Can you work these out from the model? Positions are in its coordinate system, mm. Face numbers are marked on the shaded views. A direction names the side the tool comes from. Give positions to 0.01 mm unless a question says otherwise; leave off trailing zeros. Write each loop counter-clockwise with the first axis right and the second up, starting at its lowest first coordinate (ties: lowest second). Pieces come first, ordered by that corner, then holes. Notation, with made-up numbers: (31, 23) -> (42, 23) arc R24 cw to (42, 35) -> close; hole circle Ø1 at (47.5, 84.5). An arc over 180 degrees is marked (long way). Answer as CSV lines item,"result". Start each with the question number.
1. If we section it at A-A on x = 18.5: Write out the boundary of the cut face in (y, z).
2. On a 3-axis mill with a long thin cutter (end or side, diameter ignored), from which of +Z, -Z, +X, -X, +Y, -Y can I reach the whole of each face in a straight line? I mean the marked faces 1, 2 and 3. Say none if no direction works.
3. I need wall thicknesses on line 1 (Y direction, x = 53.5, z = 4.25); line 2 (X direction, y = 33.5, z = 3.1); line 3 (Y direction, x = 41.5, z = 1.7). Which ranges of each line are inside material? Lowest first, please. Write a range as [from, to].
4. If we mould it in two halves opening along X, with no side actions, what happens to the marked faces 4, 5 and 6? For each: pulls with the +X half, pulls with the -X half, needs draft (parallel to the pull), parting line crosses it, or undercut.
5. If we section it at B-B on z = 7: Count the separate pieces of the cut face and the enclosed holes in it, plus the area to 3 significant figures.
6. I'm going to push flat-ended pins straight in: P1, Ø3, axis at x = 54.5, y = 32.5, coming from the -Z side; P2, Ø2.5, axis at x = 41.5, y = 37, coming from the +Z side; P3, Ø2.5, axis at x = 18, y = 38, coming from the +Z side. Where does each tip first touch, or does it pass through?
7. If we section it at C-C on y = 12.5: Write out the boundary of the cut face in (x, z), plus the area to 3 significant figures.
```python
from build123d import *

# Parameters (mm, degrees)
SKETCH1_W                                           = 60
SKETCH1_H                                           = 42
BOSS_EXTRUDE1_DEPTH                                 = 8
CBORE_FOR_M4_HEX_SOCKET_HEAD_CAP_SCREW2_D           = 4.5
CBORE_FOR_M4_HEX_SOCKET_HEAD_CAP_SCREW2_CBORE_D     = 8
CBORE_FOR_M4_HEX_SOCKET_HEAD_CAP_SCREW2_CBORE_DEPTH = 4.4
SKETCH4_R                                           = 2
CUT_EXTRUDE1_DEPTH                                  = 74.674961826
CBORE_FOR_M5_HEX_SOCKET_HEAD_CAP_SCREW1_D           = 5.5
CBORE_FOR_M5_HEX_SOCKET_HEAD_CAP_SCREW1_CBORE_D     = 10
CBORE_FOR_M5_HEX_SOCKET_HEAD_CAP_SCREW1_CBORE_DEPTH = 5.4
SKETCH7_R                                           = 2
CUT_EXTRUDE2_DEPTH                                  = 74.674961826
CHAMFER1_SIZE                                       = 2


with BuildPart() as part:
    # Sketch1 → Boss-Extrude1 (new body)
    with BuildSketch(Plane.XY):
        with Locations((30, 21)):
            Rectangle(SKETCH1_W, SKETCH1_H)
    extrude(amount=BOSS_EXTRUDE1_DEPTH)

    # CBORE for M4 Hex Socket Head Cap Screw2 (through all)
    with Locations(Plane.XY.offset(8)):
        with Locations((41.5, 37), (18.5, 37), (18.5, 5), (41.5, 5)):
            CounterBoreHole(CBORE_FOR_M4_HEX_SOCKET_HEAD_CAP_SCREW2_D / 2, CBORE_FOR_M4_HEX_SOCKET_HEAD_CAP_SCREW2_CBORE_D / 2, CBORE_FOR_M4_HEX_SOCKET_HEAD_CAP_SCREW2_CBORE_DEPTH)

    # Sketch4 → Cut-Extrude1 (cut, through all)
    with BuildSketch(Plane.XY.offset(8)):
        with Locations((18.5, 21)):
            Circle(SKETCH4_R)
        with Locations((41.5, 21)):
            Circle(SKETCH4_R)
    extrude(amount=-CUT_EXTRUDE1_DEPTH, mode=Mode.SUBTRACT)

    # CBORE for M5 Hex Socket Head Cap Screw1 (through all)
    with Locations(Plane(origin=(0, 0, 0), x_dir=(1, 0, 0), z_dir=(0, 0, -1))):
        with Locations((53.5, -33.5), (6.5, -33.5), (6.5, -8.5), (53.5, -8.5)):
            CounterBoreHole(CBORE_FOR_M5_HEX_SOCKET_HEAD_CAP_SCREW1_D / 2, CBORE_FOR_M5_HEX_SOCKET_HEAD_CAP_SCREW1_CBORE_D / 2, CBORE_FOR_M5_HEX_SOCKET_HEAD_CAP_SCREW1_CBORE_DEPTH)

    # Sketch7 → Cut-Extrude2 (cut, through all)
    with BuildSketch(Plane.XY.offset(8)):
        with Locations((6.5, 21)):
            Circle(SKETCH7_R)
        with Locations(Location((53.5, 21, 0), (0, 0, 180))):
            Circle(SKETCH7_R)
    extrude(amount=-CUT_EXTRUDE2_DEPTH, mode=Mode.SUBTRACT)

    # Chamfer1
    chamfer1_edges = [part.edges().sort_by_distance(p)[0] for p in [
        (0, 42, 4),
        (60, 42, 4),
        (60, 0, 4),
        (0, 0, 4),
    ]]
    chamfer(chamfer1_edges, length=CHAMFER1_SIZE)


solid = part.part
```
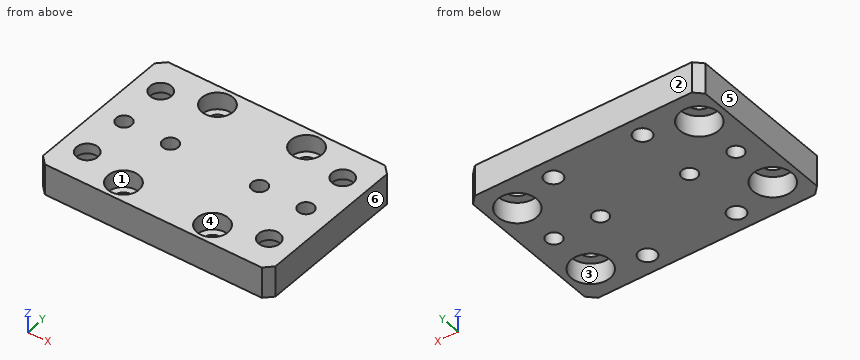
Computed values:
1,outline,"(0, 0) -> (2.75, 0) -> (2.75, 3.6) -> (1, 3.6) -> (1, 8) -> (0, 8) -> close; (7.25, 0) -> (19, 0) -> (19, 8) -> (9, 8) -> (9, 3.6) -> (7.25, 3.6) -> close; (23, 0) -> (34.75, 0) -> (34.75, 3.6) -> (33, 3.6) -> (33, 8) -> (23, 8) -> close; (39.25, 0) -> (42, 0) -> (42, 8) -> (41, 8) -> (41, 3.6) -> (39.25, 3.6) -> close"
2,face 1,"+Z"
2,face 2,"+Z, -Z, +X, -X, +Y"
2,face 3,"-Z"
3,line 1,"y = [0, 3.5], [13.5, 19], [23, 28.5], [38.5, 42]"
3,line 2,"x = [0, 1.5], [11.5, 48.5], [58.5, 60]"
3,line 3,"y = [0, 2.75], [7.25, 19], [23, 34.75], [39.25, 42]"
4,face 4,"undercut"
4,face 5,"pulls with the -X half"
4,face 6,"pulls with the +X half"
5,separate pieces,"1"
5,enclosed holes,"12"
5,area,"2,170 mm2"
6,P1,"stops at z = 5.4"
6,P2,"passes through"
6,P3,"stops at z = 3.6"
7,outline,"(0, 0) -> (3.5, 0) -> (3.5, 5.4) -> (9.5, 5.4) -> (9.5, 0) -> (50.5, 0) -> (50.5, 5.4) -> (56.5, 5.4) -> (56.5, 0) -> (60, 0) -> (60, 8) -> (0, 8) -> close"
7,area,"415 mm2"
